The figure shows three views and two pictorial views of one solid part (mm, origin at its lowest corner). Answer the questions. A direction names the side the tool comes from. Give positions to 0.01 mm unless a question says otherwise; leave off trailing zeros. Order: outer loops, then holes, each group sorted by start corner. A loop starts at its lowest first (then second) coordinate and runs counter-clockwise, first axis right, second up. Notation, with made-up numbers: (84.5, 3) -> (117.5, 3) arc R13 cw to (117.5, 23) -> close; hole circle Ø9 at (-38, 3). An arc over 180 degrees is marked (long way). One line per item, written item: value. Start each with the question number.
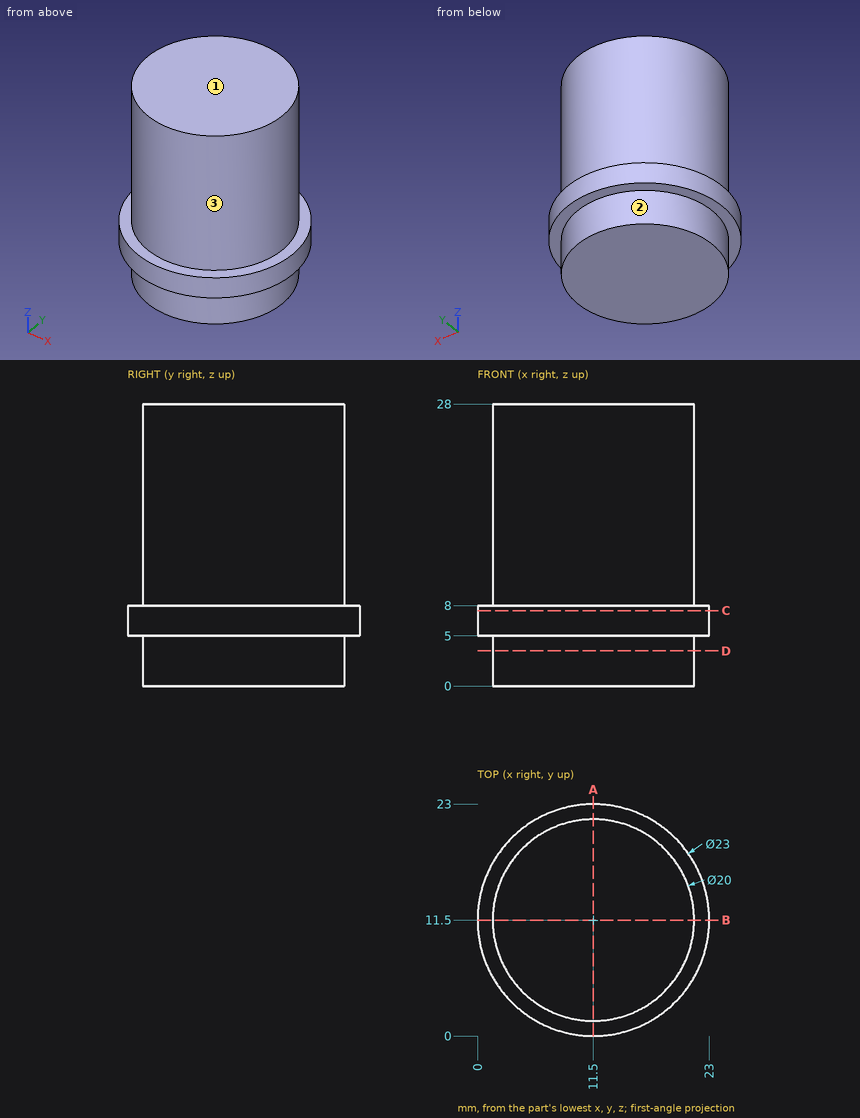
Item 1: Find section D-D on z = 3.5. Write down the section's boundary in (x, y).
Item 2: Find section A-A on x = 11.5. Write down the section's boundary in (y, z).
Item 3: Flat-ended cylindrical pins translate along their axes: pin 1 (2 mm diameter, centred on x = 3.5, z = 20.5, fed in from -Y); pin 2 (5 mm diameter, centred on x = 14, z = 18, fed in from +Y); pin 3 (12 mm diameter, centred on x = 9.5, y = 14, fed in from -Z); pin 4 (2 mm diameter, centred on x = 6, z = 7.5, fed in from +Y). Find the tip coordinate at first contact, or state that the pin passes through.
Item 4: A tool of negligible diameter and unlimited length cuts with its end or side. For the marked faces 1, 2 and 3, from which of +Z, -Z, +X, -X, +Y, -Y can it reach the whole face along a straight path? Write none if from no direction.
Item 5: Find section C-C on z = 7.5. Write down the section's boundary in (x, y), then the cut area to 3 significant figures.
Item 6: Find the intervals of material crossed by line 1 (Z direction, x = 16, y = 21); line 2 (X direction, y = 10.25, z = 24); line 3 (X direction, y = 4.5, z = 20.5), in increasing order. Write a range as from..to.
Checks:
1. outline: circle Ø20 at (11.5, 11.5)
2. outline: (0, 5) -> (1.5, 5) -> (1.5, 0) -> (21.5, 0) -> (21.5, 5) -> (23, 5) -> (23, 8) -> (21.5, 8) -> (21.5, 28) -> (1.5, 28) -> (1.5, 8) -> (0, 8) -> close
3. pin 1: y = 4.36
3. pin 2: y = 21.5
3. pin 3: z = 0
3. pin 4: y = 22.08
4. face 1: +Z, +X, -X, +Y, -Y
4. face 2: -Z
4. face 3: +Z
5. outline: circle Ø23 at (11.5, 11.5)
5. area: 415 mm2
6. line 1: 5..8
6. line 2: 1.58..21.42
6. line 3: 4.36..18.64
